Source: CAD feature listing. Evaluate the final solid. Frame: model axes, mm. A direction names the side the tool comes from. Give positions to 0.01 mm unless a question says otherwise; leave off trailing zeros. Order: outer loops, then holes, each group sorted by start corner. A loop starts at its lowest first (then second) coordinate and runs counter-clockwise, first axis right, second up. Notation, with made-up numbers: M 40.25,31.25 L 66.25,31.25 A11 ccw 66.25,47.25 Z; hole C 8.25,41.25 d5. An arc over 180 degrees is marked long. Return JSON: item names as keys, results as strings.
from build123d import *

# Parameters (mm, degrees)
SKETCH1_R           = 87.5
BOSS_EXTRUDE1_DEPTH = 800
SKETCH2_R           = 100
BOSS_EXTRUDE2_DEPTH = 700


with BuildPart() as part:
    # Sketch1 → Boss-Extrude1 (new, symmetric)
    with BuildSketch(Plane.XY):
        Circle(SKETCH1_R)
    extrude(amount=BOSS_EXTRUDE1_DEPTH, both=True)

    # Sketch2 → Boss-Extrude2 (add, symmetric)
    with BuildSketch(Plane.XY):
        Circle(SKETCH2_R)
    extrude(amount=BOSS_EXTRUDE2_DEPTH, both=True)


solid = part.part
1. First-contact query: pin 1 (4 mm diameter, centred on x = 13.5, z = 173.5, fed in from +Y); pin 2 (3 mm diameter, centred on y = -36.5, z = -375.5, fed in from +X) (3 decimals); pin 3 (3 mm diameter, centred on x = 46, z = -133, fed in from +Y). Flat tips, straight axial feed; report the tip coordinate or a pass-through.
Evaluation:
{"pin 1": "stops at y = 99.34", "pin 2": "stops at x = 93.675", "pin 3": "stops at y = 89.55"}
2. Section query A-A (x = 0). Return loops of the section in (y, z), then the cut area to 3 significant figures.
Evaluation:
{"outline": "M -100,-700 L -87.5,-700 L -87.5,-800 L 87.5,-800 L 87.5,-700 L 100,-700 L 100,700 L 87.5,700 L 87.5,800 L -87.5,800 L -87.5,700 L -100,700 Z", "area": "315,000 mm^2"}
3. Ray query, probe 1 along Y at (x, z) = (-6.5, -476); probe 2 along X at (y, z) = (-1, -585) (3 decimals); probe 3 along Z at (x, y) = (35, 85). Return the intervals inside material, ascending.
Evaluation:
{"probe 1": "y = -99.79 to 99.79", "probe 2": "x = -99.995 to 99.995", "probe 3": "z = -700 to 700"}
4. Section query C-C (z = -145). Return loops of the section in (x, y), then the cut area to 3 significant figures.
Evaluation:
{"outline": "C 0,0 d200", "area": "31,400 mm^2"}
5. Set-up query: faces 1 (the face through (-64.49, 59.14, -749.3)), 2 (the face through (-1, 1, 800)), 3 (the face through (-64.49, 59.14, 750.7)). Return all of +Z, -Z, +X, -X, +Y, -Y with unobstructed straight access to the full face (end or side cutting, diameter ignored); none if empty.
Evaluation:
{"face 1": "-Z", "face 2": "+Z, +X, -X, +Y, -Y", "face 3": "+Z"}
